CAD build for the part. Positions are in the model's coordinates, mm. Face numbers are marked on the shaded views. Give positions to 0.01 mm unless a question says otherwise; leave off trailing zeros. Write each loop counter-clockwise with the first axis right and the second up, starting at its lowest first coordinate (ties: lowest second). Pieces come first, ordered by that corner, then holes. Notation, with made-up numbers: (-8.75, 82.5) - (49.25, 82.5) arc R28 cw to (49.25, 120.5) - close; hole circle Ø10 at (-33, -12). An arc over 180 degrees is marked (long way). Answer as a JSON object with one key per item and string values.
from build123d import *

# Parameters (mm, degrees)
ROLLED_EDGE_PLATE_PROFILE_R   = 2.5
ROLLED_EDGE_PLATE_PROFILE_W   = 82
ROLLED_EDGE_PLATE_PROFILE_H   = 2
ROLLED_EDGE_PLATE_PROFILE_W_2 = 1
ROLLED_EDGE_PLATE_PROFILE_W_3 = 8
PLATE_EXTRUDE_35MM_DEPTH      = 17.5
EDGE_FILLETS_R0_5_R           = 0.5


with BuildPart() as part:
    # Rolled Edge Plate Profile → Plate Extrude 35mm (new, symmetric)
    # profile 1 of 7: a face of its own
    with BuildSketch(Plane.XY):
        with BuildLine():
            Line((41, 5), (41, 1))
            Line((41, 1), (49, 1))
            Line((49, 1), (49, 5))
            ThreePointArc((49, 5), (45, 9), (41, 5))
        make_face()
        with Locations((45, 5)):
            Circle(ROLLED_EDGE_PLATE_PROFILE_R, mode=Mode.SUBTRACT)
    # profile 2 of 7: a face of its own
    with BuildSketch(Plane.XY):
        Rectangle(ROLLED_EDGE_PLATE_PROFILE_W, ROLLED_EDGE_PLATE_PROFILE_H)
    # profile 3 of 7: a face of its own
    with BuildSketch(Plane.XY):
        with Locations((49.5, 0)):
            Rectangle(ROLLED_EDGE_PLATE_PROFILE_W_2, ROLLED_EDGE_PLATE_PROFILE_H)
    # profile 4 of 7: a face of its own
    with BuildSketch(Plane.XY):
        with Locations((45, 0)):
            Rectangle(ROLLED_EDGE_PLATE_PROFILE_W_3, ROLLED_EDGE_PLATE_PROFILE_H)
    # profile 5 of 7: a face of its own
    with BuildSketch(Plane.XY):
        with Locations((-45, 0)):
            Rectangle(ROLLED_EDGE_PLATE_PROFILE_W_3, ROLLED_EDGE_PLATE_PROFILE_H)
    # profile 6 of 7: a face of its own
    with BuildSketch(Plane.XY):
        with Locations((-49.5, 0)):
            Rectangle(ROLLED_EDGE_PLATE_PROFILE_W_2, ROLLED_EDGE_PLATE_PROFILE_H)
    # profile 7 of 7: a face of its own
    with BuildSketch(Plane.XY):
        with BuildLine():
            Line((-49, 5), (-49, 1))
            Line((-49, 1), (-41, 1))
            Line((-41, 1), (-41, 5))
            ThreePointArc((-41, 5), (-45, 9), (-49, 5))
        make_face()
        with Locations((-45, 5)):
            Circle(ROLLED_EDGE_PLATE_PROFILE_R, mode=Mode.SUBTRACT)
    extrude(amount=PLATE_EXTRUDE_35MM_DEPTH, both=True)

    # Edge Fillets R0.5
    edge_fillets_r0_5_edges = [part.edges().sort_by_distance(p)[0] for p in [
        (50, 1, 0),
        (50, -1, 0),
        (-50, -1, 0),
        (-50, 1, 0),
    ]]
    fillet(edge_fillets_r0_5_edges, radius=EDGE_FILLETS_R0_5_R)


solid = part.part
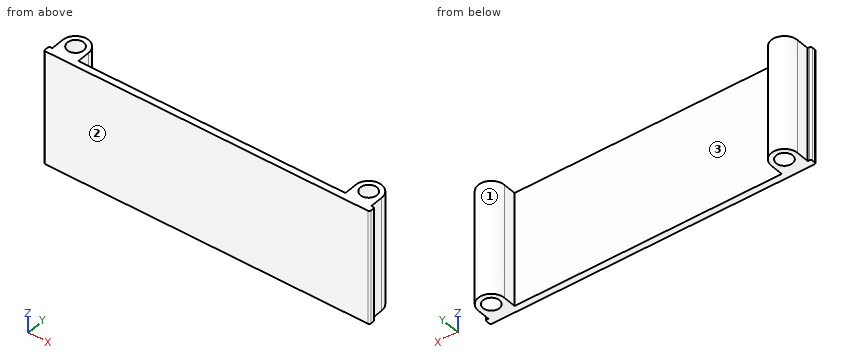
Item 1: Cut at C-C (z = -6). Give the cut face in (x, y).
Entries:
{"outline": "(-50, -0.5) arc R0.5 ccw to (-49.5, -1) - (49.5, -1) arc R0.5 ccw to (50, -0.5) - (50, 0.5) arc R0.5 ccw to (49.5, 1) - (49, 1) - (49, 5) arc R4 ccw to (41, 5) - (41, 1) - (-41, 1) - (-41, 5) arc R4 ccw to (-49, 5) - (-49, 1) - (-49.5, 1) arc R0.5 ccw to (-50, 0.5) - close; hole circle Ø5 at (-45, 5); hole circle Ø5 at (45, 5)"}
Item 2: Cut at B-B (y = 3.5). Give the cut face in (x, z).
Entries:
{"outline": "(-49, -17.5) - (-47, -17.5) - (-47, 17.5) - (-49, 17.5) - close; (-43, -17.5) - (-41, -17.5) - (-41, 17.5) - (-43, 17.5) - close; (41, -17.5) - (43, -17.5) - (43, 17.5) - (41, 17.5) - close; (47, -17.5) - (49, -17.5) - (49, 17.5) - (47, 17.5) - close"}
Item 3: Probe line 1 (X direction, y = 2.25, z = -5); line 2 (Y direction, x = -45, z = 1.5); line 3 (X direction, y = 5.5, z = -7.5). List the from-to ranges inside material, lowest first. Write a range as from..to.
Entries:
{"line 1": "-49..-41, 41..49", "line 2": "-1..2.5, 7.5..9", "line 3": "-48.97..-47.45, -42.55..-41.03, 41.03..42.55, 47.45..48.97"}
Item 4: Cut at A-A (x = -45). Give the cut face in (y, z).
Entries:
{"outline": "(-1, -17.5) - (2.5, -17.5) - (2.5, 17.5) - (-1, 17.5) - close; (7.5, -17.5) - (9, -17.5) - (9, 17.5) - (7.5, 17.5) - close"}
Item 5: Mould opens along X. For the marked faces 1, 2 and 3 say: +X half, -X half, draft (parallel to the pull), parting line (faces both ways), or undercut.
Entries:
{"face 1": "undercut", "face 2": "draft", "face 3": "undercut"}
Item 6: Flat gauge pins, fed straight in: P1, Ø3, axis at y = 3, z = -7.5, coming from the -X side; P2, Ø5, axis at x = 5, z = 9, coming from the +Y side; P3, Ø3, axis at x = 45, y = 5, coming from the -Z side; P4, Ø1.2, axis at y = 3, z = 6.5, coming from the +X side. Where does each tip first touch, or does it go through?
Entries:
{"P1": "x = -49", "P2": "y = 1", "P3": "through", "P4": "x = 49"}
Item 7: Cut at D-D (x = -24.5). Give the cut face in (y, z).
Entries:
{"outline": "(-1, -17.5) - (1, -17.5) - (1, 17.5) - (-1, 17.5) - close"}
